CAD build for the part. Positions are in the model's coordinates, mm. A direction names the side the tool comes from. Give positions to 0.01 mm unless a question says otherwise; leave off trailing zeros. Loops run counter-clockwise (first coordinate to the right, second up) from the corner with the lowest first, then second, coordinate; pieces in that order, holes last.
```python
from build123d import *

# Parameters (mm, degrees)
SKETCH1_W           = 20
SKETCH1_H           = 30
SKETCH1_W_2         = 18
SKETCH1_H_2         = 28
BOSS_EXTRUDE1_DEPTH = 859
BOSS_EXTRUDE2_DEPTH = 1
SKETCH4_R           = 5
CUT_EXTRUDE1_DEPTH  = 890.778062216
SKETCH5_R           = 4
CUT_EXTRUDE2_DEPTH  = 890.753898558
SKETCH6_W           = 20
SKETCH6_H           = 30
SKETCH6_W_2         = 18
SKETCH6_H_2         = 28
BOSS_EXTRUDE3_DEPTH = 300


with BuildPart() as part:
    # Sketch1 → Boss-Extrude1 (new body)
    with BuildSketch(Plane.XY):
        with Locations((10, -15)):
            Rectangle(SKETCH1_W, SKETCH1_H)
        with Locations((10, -15)):
            Rectangle(SKETCH1_W_2, SKETCH1_H_2, mode=Mode.SUBTRACT)
    extrude(amount=BOSS_EXTRUDE1_DEPTH)

    # Sketch3 → Boss-Extrude2 (add)
    with BuildSketch(Plane.ZY):
        with BuildLine():
            Line((829, -30), (859, -30))
            Line((859, -30), (886, -30))
            ThreePointArc((886, -30), (888.121320344, -29.121320344), (889, -27))
            Line((889, -27), (889, -3))
            ThreePointArc((889, -3), (888.121320344, -0.878679656), (886, 0))
            Line((886, 0), (859, 0))
            Line((859, 0), (829, 0))
            Line((829, 0), (829, -30))
        make_face()
    boss_extrude2 = extrude(amount=BOSS_EXTRUDE2_DEPTH)

    # Mirror2: Boss-Extrude2 across plane
    add(boss_extrude2.mirror(Plane(origin=(10, 0, 0), x_dir=(0, 0, 1), z_dir=(1, 0, 0))))

    # Sketch4 → Cut-Extrude1 (cut, through all)
    with BuildSketch(Plane(origin=(21, 0, 0), x_dir=(0, 0, -1), z_dir=(1, 0, 0))):
        with Locations(Location((-877.5, -15, 0), (0, 0, 90))):
            Circle(SKETCH4_R)
    extrude(amount=-CUT_EXTRUDE1_DEPTH, mode=Mode.SUBTRACT)

    # Sketch5 → Cut-Extrude2 (cut, through all)
    with BuildSketch(Plane(origin=(0, 0, 0), x_dir=(1, 0, 0), z_dir=(0, 1, 0))):
        with Locations(Location((10, -144, 0), (0, 0, 270))):
            Circle(SKETCH5_R)
        with Locations(Location((10, -432, 0), (0, 0, 270))):
            Circle(SKETCH5_R)
        with Locations(Location((10, -720, 0), (0, 0, 270))):
            Circle(SKETCH5_R)
    extrude(amount=-CUT_EXTRUDE2_DEPTH, mode=Mode.SUBTRACT)

    # Sketch6 → Boss-Extrude3 (add)
    with BuildSketch(Plane(origin=(0, 0, 0), x_dir=(-1, 0, 0), z_dir=(0, 0, -1))):
        with Locations((-10, -15)):
            Rectangle(SKETCH6_W, SKETCH6_H)
        with Locations((-10, -15)):
            Rectangle(SKETCH6_W_2, SKETCH6_H_2, mode=Mode.SUBTRACT)
    extrude(amount=BOSS_EXTRUDE3_DEPTH)


solid = part.part
```
1. Tool access for faces 1 (the face through (19, -15, 288)), 2 (the face through (0, -15, 272)), 3 (the face through (20, -15, 272)): list every direction of +Z, -Z, +X, -X, +Y, -Y with a clear straight run to the whole face (end or side of a thin tool).
Responses:
face 1: +Z, -Z
face 2: -Z, -X, +Y, -Y
face 3: -Z, +X, +Y, -Y
2. Probe line 1 along Y through (x, z) = (16, 646.5); line 2 along X through (y, z) = (-10.5, 290.5); line 3 along X through (y, z) = (-0.25, 432). List the from-to ranges inside material, lowest first.
Responses:
line 1: y = -30 to -29, -1 to 0
line 2: x = 0 to 1, 19 to 20
line 3: x = 0 to 6, 14 to 20
3. Saw through at B-B, the plane x = 10. Count the separate pieces of the cut face and the enclosed holes in it, and give its area (3 significant figures).
Responses:
separate pieces: 8
enclosed holes: 0
area: 2,270 mm2
4. Saw through at A-A, the plane y = -15. List the corners of the cut face in (x, z).
Responses:
outline: (-1, 829) - (0, 829) - (0, -300) - (1, -300) - (1, 859) - (0, 859) - (0, 872.5) - (-1, 872.5) - close; (-1, 882.5) - (0, 882.5) - (0, 889) - (-1, 889) - close; (19, -300) - (20, -300) - (20, 829) - (21, 829) - (21, 872.5) - (20, 872.5) - (20, 859) - (19, 859) - close; (20, 882.5) - (21, 882.5) - (21, 889) - (20, 889) - close
5. Pull direction Y, two halves, no side cores. Call faces 4 (the face through (-1, -15, 859)), 5 (the face through (10, -30, 301)), 6 (the face through (10, -1, 288)): released by +Y, released by -Y, zero draft, split by the parting line, or undercut.
Responses:
face 4: zero draft
face 5: released by -Y
face 6: undercut
6. Drop flat-ended pins along their axis: pin 1 (0.5 mm diameter, centred on x = 20.5, y = -9, fed in from -Z); pin 2 (10 mm diameter, centred on y = -15.5, z = -104, fed in from -X); pin 3 (6 mm diameter, centred on x = 18, z = -71.5, fed in from +Y); pin 4 (12 mm diameter, centred on y = -8, z = -33.5, fed in from +X). Give the stop position or say it passes through.
Responses:
pin 1: stops at z = 829
pin 2: stops at x = 0
pin 3: stops at y = 0
pin 4: stops at x = 20
7. Saw through at C-C, the plane z = 574.5. List the corners of the cut face in (x, y).
Responses:
outline: (0, -30) - (20, -30) - (20, 0) - (0, 0) - close; hole (1, -29) - (19, -29) - (19, -1) - (1, -1) - close
